The model under review builds one solid part; all positions refer to its coordinate system, in mm. A direction names the side the tool comes from. Give positions to 0.01 mm unless a question says otherwise; leave off trailing zeros. Answer as a JSON object with one key per item and string values.
from build123d import *

# Parameters (mm, degrees)
BOSS_EXTRUDE1_DEPTH = 2660


with BuildPart() as part:
    # Sketch1 → Boss-Extrude1 (new body)
    with BuildSketch(Plane.XY):
        with BuildLine():
            Line((0, 0), (0, 38))
            ThreePointArc((0, 38), (-3.514718626, 46.485281374), (-12, 50))
            Line((-12, 50), (-59, 50))
            ThreePointArc((-59, 50), (-63.242640687, 51.757359313), (-65, 56))
            Line((-65, 56), (-65, 91))
            ThreePointArc((-65, 91), (-68.514718626, 99.485281374), (-77, 103))
            Line((-77, 103), (-162, 103))
            ThreePointArc((-162, 103), (-170.485281374, 99.485281374), (-174, 91))
            Line((-174, 91), (-174, 21))
            ThreePointArc((-174, 21), (-170.485281374, 12.514718626), (-162, 9))
            Line((-162, 9), (-127, 9))
            ThreePointArc((-127, 9), (-122.757359313, 7.242640687), (-121, 3))
            Line((-121, 3), (-121, -43))
            ThreePointArc((-121, -43), (-117.485281374, -51.485281374), (-109, -55))
            Line((-109, -55), (-71, -55))
            Line((-71, -55), (-71, -49))
            Line((-71, -49), (-109, -49))
            ThreePointArc((-109, -49), (-113.242640687, -47.242640687), (-115, -43))
            Line((-115, -43), (-115, 3))
            ThreePointArc((-115, 3), (-118.514718626, 11.485281374), (-127, 15))
            Line((-127, 15), (-162, 15))
            ThreePointArc((-162, 15), (-166.242640687, 16.757359313), (-168, 21))
            Line((-168, 21), (-168, 91))
            ThreePointArc((-168, 91), (-166.242640687, 95.242640687), (-162, 97))
            Line((-162, 97), (-77, 97))
            ThreePointArc((-77, 97), (-72.757359313, 95.242640687), (-71, 91))
            Line((-71, 91), (-71, 56))
            ThreePointArc((-71, 56), (-67.485281374, 47.514718626), (-59, 44))
            Line((-59, 44), (-12, 44))
            ThreePointArc((-12, 44), (-7.757359313, 42.242640687), (-6, 38))
            Line((-6, 38), (-6, 0))
            Line((-6, 0), (0, 0))
        make_face()
    extrude(amount=BOSS_EXTRUDE1_DEPTH)


solid = part.part
Q1. To check wall thickness, follow probe 1 along Y at (x, z) = (-88, 847); probe 2 along Y at (x, z) = (-141, 1257.5); probe 3 along X at (y, z) = (59, 1360). State the ranges of each line that lie inside material, in increasing order. Write a range as [from, to].
Results:
{"probe 1": "y = [-55, -49], [97, 103]", "probe 2": "y = [9, 15], [97, 103]", "probe 3": "x = [-174, -168], [-71, -65]"}
Q2. For faces 5 (the face through (-126, 13, 2660)), 6 (the face through (-36, 44, 1311)), 7 (the face through (-35, 50, 1311)), list the 3-axis set-ups (+Z, -Z, +X, -X, +Y, -Y) from which the entire face can be reached by the end or side of a thin tool; tool diameter is ignored.
Results:
{"face 5": "+Z, +X, -X, +Y, -Y", "face 6": "+Z, -Z, -Y", "face 7": "+Z, -Z, +X, +Y"}
Q3. The part is to be moulded in two halves that separate along X. For faces 1 (the face through (-168, 56, 1311)), 2 (the face through (-121, -20, 1311)), 3 (the face through (-120, 97, 1311)), 4 (the face through (-119, 103, 1311)), say which applies: +X half, -X half, draft (parallel to the pull), parting line (faces both ways), or undercut.
Results:
{"face 1": "undercut", "face 2": "-X half", "face 3": "undercut", "face 4": "draft"}
Q4. Clearance check with flat-ended pins moving along their axes: pin 1 Ø4 at (y, z) = (47.5, 1170) entering from +X; pin 2 Ø1.8 at (y, z) = (-53, 1009) entering from +X; pin 3 Ø10.5 at (x, z) = (-143.5, 1929) entering from -Y. State where each tip first meets the part, or that it passes through.
Results:
{"pin 1": "stops at x = -2.63", "pin 2": "stops at x = -71", "pin 3": "stops at y = 9"}
